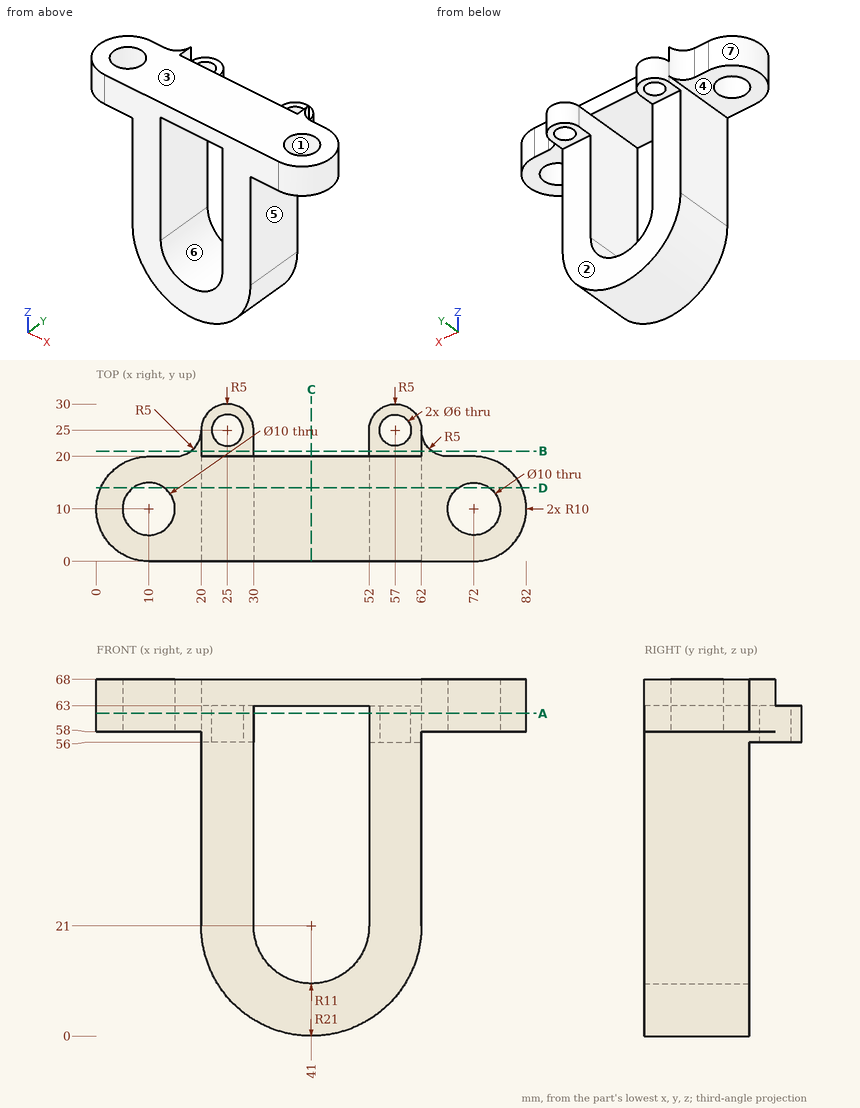
Answer from the drawing. Dimensions are ordinates in mm from the lowest x, y and z of the part. A direction names the side the tool comes from. Give positions to 0.01 mm unless a question says otherwise; leave off trailing zeros. Loops run counter-clockwise (first coordinate to the right, second up) from the corner with the lowest first, then second, coordinate; pieces in that order, holes last. Notation, with made-up numbers: M 13,24.25 L 55,24.25 A18 ccw 55,43.25 Z; hole C 75,20 d5. An arc over 180 degrees is marked long. One line per item, written item: value.
Q1. Determine the mould class of the marked faces 1, 2 and 3 for opening direction Y: +Y half, -Y half, draft (parallel to the pull), parting line (faces both ways), or undercut.
Working result:
face 1: undercut
face 2: +Y half
face 3: draft
Q2. A cutting plane is placed at D-D on y = 14. Determine the outline of the cut face in (x, z).
Working result:
outline: M 0.83,58 L 7,58 L 7,68 L 0.83,68 Z; M 13,58 L 20,58 L 20,21 A21 ccw 62,21 L 62,58 L 69,58 L 69,68 L 13,68 Z; M 75,58 L 81.17,58 L 81.17,68 L 75,68 Z; hole M 30,21 A11 ccw 52,21 L 52,63 L 30,63 Z
Q3. Find the intervals of material crossed by line 1 (Y direction, x = 57, z = 60.25); line 2 (Y direction, x = 72, z = 62); line 3 (Z direction, x = 41.5, y = 5.5), in increasing order. Write a range as from..to.
Working result:
line 1: y = 0..22, 28..30
line 2: y = 0..5, 15..20
line 3: z = 0.01..10.01, 63..68
Q4. A cutting plane is placed at C-C on x = 41. Determine the outline of the cut face in (y, z).
Working result:
outline: M 0,0 L 20,0 L 20,10 L 0,10 Z; M 0,63 L 20,63 L 20,68 L 0,68 Z
Q5. For the marked faces 4, 5, 6 and 7, determine the directions among +Z, -Z, +X, -X, +Y, -Y from which every point of the face is accessible in a straight line to the end or side of a thin tool.
Working result:
face 4: -Z, -X, +Y, -Y
face 5: -Z, +X, +Y, -Y
face 6: +Y, -Y
face 7: +Z, -Z, -X
Q6. Flat-ended cylindrical pins translate along their axes: P1, Ø1, axis at x = 9, y = 7.5, coming from the +Z side; P2, Ø5, axis at x = 73, y = 4.5, coming from the -Z side; P3, Ø12, axis at y = 22.5, z = 49, coming from the -X side; P4, Ø7.5, axis at y = 7, z = 49.5, coming from the +X side. Find the tip coordinate at first contact, or state that the pin passes through.
Working result:
P1: passes through
P2: stops at z = 58
P3: stops at x = 20
P4: stops at x = 62
Q7. A cutting plane is placed at B-B on y = 21. Determine the outline of the cut face in (x, z).
Working result:
outline: M 18,58 L 20,58 L 20,56 L 30,56 L 30,63 L 20,63 L 20,68 L 18,68 Z; M 52,56 L 62,56 L 62,58 L 64,58 L 64,68 L 62,68 L 62,63 L 52,63 Z
Q8. A cutting plane is placed at A-A on z = 61.5. Determine the outline of the cut face in (x, y), then the cut area to 3 significant figures.
Working result:
outline: M 10,0 L 30,0 L 30,25 A5 ccw 20,25 A5 cw 15,20 L 10,20 A10 ccw Z; M 52,0 L 72,0 A10 ccw 72,20 L 67,20 A5 cw 62,25 A5 ccw 52,25 Z; hole C 10,10 d10; hole C 25,25 d6; hole C 57,25 d6; hole C 72,10 d10
area: 1,090 mm^2
